Can you work these out from the drawing? Everything is in mm from the part's minimum corner. A direction names the side the tool comes from. Coordinates: 2 decimals unless noted, no trailing zeros. Order: outer loops, then holes, each group sorted by start corner. A loop starts at its lowest first (then second) coordinate and runs counter-clockwise, first axis right, second up. Notation, with made-up numbers: M 52,-23.75 L 104,-23.75 A27 ccw 104,4.25 Z; hole C -3.5,49.5 d9. An arc over 180 degrees is marked long. Answer as a JSON object with one key per item and string values.
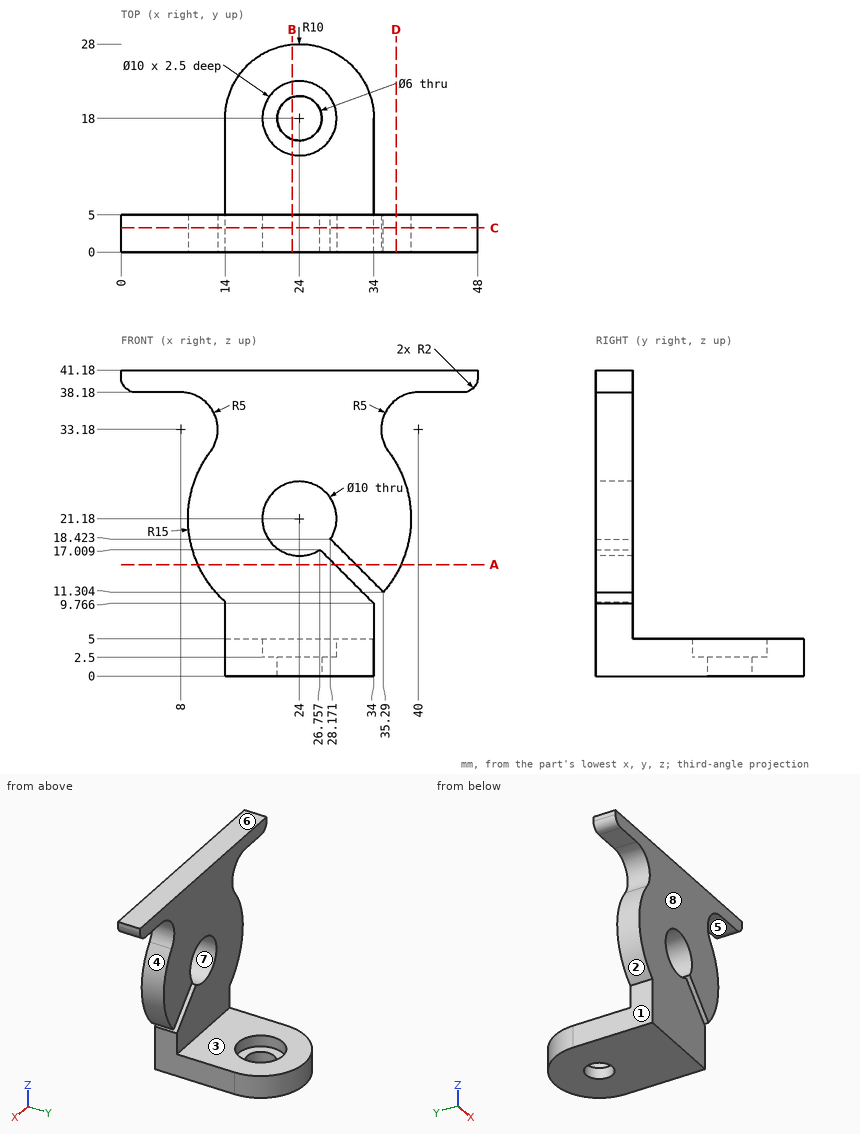
Item 1: I want a section at B-B, the plane x = 23. Write out the boundary of the cut face in (y, z).
Answers follow:
{"outline": "M 0,0 L 15.17,0 L 15.17,2.5 L 13.1,2.5 L 13.1,5 L 5,5 L 5,16.28 L 0,16.28 Z; M 0,26.08 L 5,26.08 L 5,41.18 L 0,41.18 Z; M 20.83,0 L 27.95,0 L 27.95,5 L 22.9,5 L 22.9,2.5 L 20.83,2.5 Z"}
Item 2: I want a section at D-D, the plane x = 37. Write out the boundary of the cut face in (y, z).
Answers follow:
{"outline": "M 0,13.7 L 5,13.7 L 5,28.66 L 0,28.66 Z; M 0,37.18 L 5,37.18 L 5,41.18 L 0,41.18 Z"}
Item 3: I'm going to push flat-ended pins straight in: pin 1 (3 mm diameter, centred on y = 7, z = 14, fed in from +X); pin 2 (11 mm diameter, centred on x = 16, z = 28.5, fed in from +Y); pin 3 (8 mm diameter, centred on x = 9, y = 5, fed in from -Z); pin 4 (10.5 mm diameter, centred on y = 6.5, z = 5.5, fed in from +X). Where does each tip first touch, or does it pass through?
Answers follow:
{"pin 1": "passes through", "pin 2": "stops at y = 5", "pin 3": "stops at z = 10.98", "pin 4": "stops at x = 34"}
Item 4: Please list where these lines run through material, in increasing order: line 1 (Y direction, x = 24, z = 1.7); line 2 (Z direction, x = 24, y = 3.5); line 3 (Y direction, x = 24, z = 3).
Answers follow:
{"line 1": "y = 0 to 15, 21 to 28", "line 2": "z = 0 to 16.18, 26.18 to 41.18", "line 3": "y = 0 to 13, 23 to 28"}
Item 5: I want a section at A-A, the plane z = 15. Write out the boundary of the cut face in (x, y) (1 decimal).
Answers follow:
{"outline": "M 10.3,0 L 28.8,0 L 28.8,5 L 10.3,5 Z; M 31.6,0 L 37.7,0 L 37.7,5 L 31.6,5 Z"}
Item 6: I want a section at C-C, the plane y = 3.25. Write out the boundary of the cut face in (x, z) (1 decimal), plus the area to 3 significant figures.
Answers follow:
{"outline": "M 0,40.2 A2 ccw 2,38.2 L 8,38.2 A5 cw 12,30.2 A15 ccw 14,10 L 14,0 L 34,0 L 34,9.8 L 26.8,17 A5 cw long 28.2,18.4 L 35.3,11.3 A15 ccw 36,30.2 A5 cw 40,38.2 L 46,38.2 A2 ccw 48,40.2 L 48,41.2 L 0,41.2 Z", "area": "986 mm^2"}
Item 7: Which directions (+Z, -Z, +X, -X, +Y, -Y) give clear straight access to the entire face, cutting with the end or side of a thin tool? Please do the marked faces 1, 2, 3, 4 and 5.
Answers follow:
{"face 1": "-Z, -X, +Y, -Y", "face 2": "-X, +Y, -Y", "face 3": "+Z, +X, -X, +Y", "face 4": "+X, +Y, -Y", "face 5": "-Z, +X, +Y, -Y"}
Item 8: If we mould it in two halves opening along Z, with no side actions, what happens to the marked faces 6, 7 and 8? For each: pulls with the +Z half, pulls with the -Z half, needs draft (parallel to the pull), parting line crosses it, or undercut.
Answers follow:
{"face 6": "pulls with the +Z half", "face 7": "undercut", "face 8": "needs draft"}
